```python
from build123d import *

# Parameters (mm, degrees)
BRACKET_BODY_DEPTH           = 42
UPRIGHT_TOP_ROUND_R20_R      = 20
SUPPORT_RIB_REACH            = 146.156
SUPPORT_RIB_SKETCH_WALL_W    = 387.75542236
SUPPORT_RIB_SKETCH_WALL_H    = 24
BASE_MOUNTING_HOLES_REACH    = 106.828
BASE_MOUNTING_HOLES_SKETCH_R = 10
UPRIGHT_HOLE_20_REACH        = 157.769
UPRIGHT_HOLE_SKETCH_R        = 10


with BuildPart() as part:
    # Bracket Profile Sketch → Bracket Body (new, symmetric)
    with BuildSketch(Plane.XY):
        Polygon((-75, 90), (-75, 0), (75, 0), (75, 10), (40.358983849, 30), (-45, 30), (-45, 90), align=None)
    extrude(amount=BRACKET_BODY_DEPTH, both=True)

    # Upright Top Round R20
    upright_top_round_r20_edges = [part.edges().sort_by_distance(p)[0] for p in [
        (-60, 90, 42),
    ]]
    fillet(upright_top_round_r20_edges, radius=UPRIGHT_TOP_ROUND_R20_R)

    # Support Rib Sketch wall → Support Rib (add, up to next)
    with BuildSketch(Plane(origin=(-2.320508076, 53.5, -42), x_dir=(-0.875988049468, 0.482332807497, 0), z_dir=(0.482332807497, 0.875988049468, 0)), mode=Mode.PRIVATE) as support_rib_sk1:
        with Locations((0, 12)):
            Rectangle(SUPPORT_RIB_SKETCH_WALL_W, SUPPORT_RIB_SKETCH_WALL_H)
    support_rib_tool1 = extrude(support_rib_sk1.sketch, amount=-SUPPORT_RIB_REACH, mode=Mode.PRIVATE) - part.part
    add(support_rib_tool1.solids().sort_by_distance((-2.320508076, 53.5, -42))[0])

    # Base Mounting Holes Sketch → Base Mounting Holes (cut, up to next)
    with BuildSketch(Plane(origin=(0, 30, 0), x_dir=(1, 0, 0), z_dir=(0, 1, 0)), mode=Mode.PRIVATE) as base_mounting_holes_sk1:
        with Locations(Location((-25, -22, 0), (0, 0, 180))):
            Circle(BASE_MOUNTING_HOLES_SKETCH_R)
    base_mounting_holes_tool1 = extrude(base_mounting_holes_sk1.sketch, amount=-BASE_MOUNTING_HOLES_REACH, mode=Mode.PRIVATE) & part.part
    # Base Mounting Holes Sketch → Base Mounting Holes (cut, up to next)
    with BuildSketch(Plane(origin=(0, 30, 0), x_dir=(1, 0, 0), z_dir=(0, 1, 0)), mode=Mode.PRIVATE) as base_mounting_holes_sk2:
        with Locations(Location((20, -22, 0), (0, 0, 180))):
            Circle(BASE_MOUNTING_HOLES_SKETCH_R)
    base_mounting_holes_tool2 = extrude(base_mounting_holes_sk2.sketch, amount=-BASE_MOUNTING_HOLES_REACH, mode=Mode.PRIVATE) & part.part
    add(base_mounting_holes_tool1.solids().sort_by_distance((-25, 30, 22))[0], mode=Mode.SUBTRACT)
    add(base_mounting_holes_tool2.solids().sort_by_distance((20, 30, 22))[0], mode=Mode.SUBTRACT)

    # Upright Hole Sketch → Upright Hole Ø20 (cut, up to next)
    with BuildSketch(Plane(origin=(-45, 0, 0), x_dir=(0, 0, -1), z_dir=(1, 0, 0)), mode=Mode.PRIVATE) as upright_hole_20_sk1:
        with Locations((-22, 70)):
            Circle(UPRIGHT_HOLE_SKETCH_R)
    upright_hole_20_tool1 = extrude(upright_hole_20_sk1.sketch, amount=-UPRIGHT_HOLE_20_REACH, mode=Mode.PRIVATE) & part.part
    add(upright_hole_20_tool1.solids().sort_by_distance((-45, 70, 22))[0], mode=Mode.SUBTRACT)


solid = part.part
```
For this review, take the finished solid that the model builds, in its own axes (mm). A direction names the side the tool comes from. Round coordinates to 2 decimals unless told otherwise and drop trailing zeros. Loops run counter-clockwise (first coordinate to the right, second up) from the corner with the lowest first, then second, coordinate; pieces in that order, holes last.
(1) We need section C-C (y = 13.5). Give the boundary of the cut face in (x, z).
Returned:
outline: (-75, -42) - (68.94, -42) - (68.94, 42) - (-75, 42) - close; hole circle Ø20 at (-25, 22); hole circle Ø20 at (20, 22)
(2) Mouldability with a two-part tool opening along Z and no side actions: class faces 1 (the cylindrical face through (-34.54, 15.21, 25)), 2 (the cylindrical face through (-59.79, 78.43, 16.62)), 3 (the flat face through (-2, 30, 12)), 4 (the flat face through (-18, 20, 42)) as released by +Z, released by -Z, zero draft, split by the parting line, or undercut.
Returned:
face 1: undercut
face 2: undercut
face 3: zero draft
face 4: released by +Z
(3) Tool access review of faces 5 (the cylindrical face through (-60.21, 84.297, 35.986)), 6 (the flat face through (-17, 49, -18)): name each direction out of +Z, -Z, +X, -X, +Y, -Y from which nothing blocks a thin tool from reaching the whole face with its end or side.
Returned:
face 5: +Z, +X, -X, +Y
face 6: +Z, +X, +Y
(4) We need section A-A (z = -28). Give the boundary of the cut face in (x, y), plus the area to 3 significant figures.
Returned:
outline: (-75, 0) - (75, 0) - (75, 10) - (40.36, 30) - (-45, 77) - (-45, 90) - (-75, 90) - close
area: 7,960 mm2
(5) We need section D-D (y = 52). Give the boundary of the cut face in (x, z), plus the area to 3 significant figures.
Returned:
outline: (-75, -42) - (0.4, -42) - (0.4, -18) - (-45, -18) - (-45, 42) - (-75, 42) - close
area: 3,610 mm2
(6) Clearance check with flat-ended pins moving along their axes: P1, Ø3, axis at x = -9.5, z = -25.5, coming from the +Y side; P2, Ø14, axis at x = -1.5, y = 55.5, coming from the +Z side; P3, Ø23, axis at x = -25, z = 22, coming from the -Y side; P4, Ø5, axis at y = 53, z = 28.5, coming from the +X side. State where each tip first meets the part, or that it passes through.
Returned:
P1: stops at y = 58.28
P2: stops at z = -18
P3: stops at y = 0
P4: stops at x = -45
(7) We need section B-B (x = 22.5). Give the boundary of the cut face in (y, z), plus the area to 3 significant figures.
Returned:
outline: (0, -42) - (39.83, -42) - (39.83, -18) - (30, -18) - (30, 12.32) - (0, 12.32) - close; (0, 31.68) - (30, 31.68) - (30, 42) - (0, 42) - close
area: 2,180 mm2
(8) Wall thickness on line 1 along Z through (x, y) = (-25, 16); line 2 along Z through (x, y) = (-31, 39.5); line 3 along Y through (x, z) = (-2.5, 36.5): over which ranges is each line inside the solid? List them lowest first.
Returned:
line 1: z = -42 to 12, 32 to 42
line 2: z = -42 to -18
line 3: y = 0 to 30
